from build123d import *

# Parameters (mm, degrees)
SKETCH_1_W          = 130
SKETCH_1_H          = 130
EXTRUDE_1_DEPTH     = 8
SKETCH_2_W          = 116
SKETCH_2_H          = 116
EXTRUDE_2_DEPTH     = 54
SKETCH_3_W          = 114.015684478
SKETCH_3_H          = 114.394474128
CUT_EXTRUDE_1_DEPTH = 2


with BuildPart() as part:
    # 草图1 → 凸台-拉伸1 (new body)
    with BuildSketch(Plane(origin=(0, 0, 0), x_dir=(0, 0, -1), z_dir=(1, 0, 0))):
        Rectangle(SKETCH_1_W, SKETCH_1_H)
    extrude(amount=EXTRUDE_1_DEPTH)

    # 草图2 → 凸台-拉伸2 (add)
    with BuildSketch(Plane(origin=(8, 0, 0), x_dir=(0, 0, -1), z_dir=(1, 0, 0))):
        Rectangle(SKETCH_2_W, SKETCH_2_H)
    extrude(amount=EXTRUDE_2_DEPTH)

    # 草图3 → 切除-拉伸1 (cut)
    with BuildSketch(Plane.ZY):
        Rectangle(SKETCH_3_W, SKETCH_3_H)
    extrude(amount=-CUT_EXTRUDE_1_DEPTH, mode=Mode.SUBTRACT)


solid = part.part
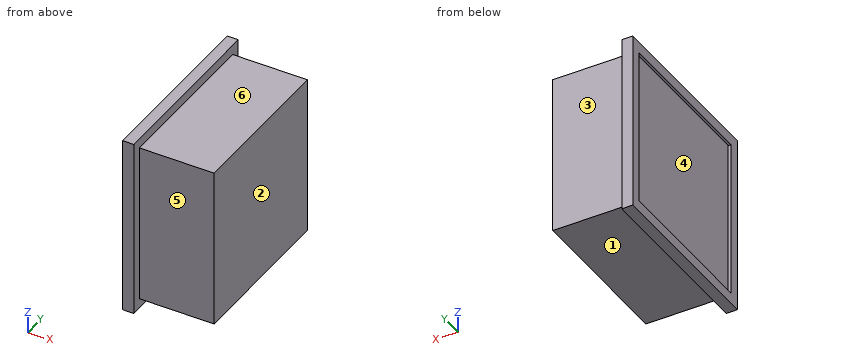
Here's how the part is built. I have some questions about the finished solid (model axes, mm). Face numbers are marked on the shaded views. A direction names the side the tool comes from. Coordinates: 2 decimals unless noted, no trailing zeros. Order: outer loops, then holes, each group sorted by start corner. A loop starts at its lowest first (then second) coordinate and runs counter-clockwise, first axis right, second up. Notation, with made-up numbers: M 83,59.5 L 131,59.5 A22 ccw 131,83.5 Z; hole C 30.5,71.25 d6. An arc over 180 degrees is marked long. Answer as CSV lines item,"result".
Item 1: If I drill on line 1 (Y direction, x = 32, z = -12.5); line 2 (X direction, y = 42, z = 32.5), over which ranges is the centre line in solid material (lowest first)?
Results found:
line 1,"-58 to 58"
line 2,"2 to 62"
Item 2: Imagine slicing it at C-C on x = 31. Write out the boundary of the cut face in (y, z), plus the area to 3 significant figures.
Results found:
outline,"M -58,-58 L 58,-58 L 58,58 L -58,58 Z"
area,"13,500 mm2"
Item 3: Imagine slicing it at B-B on y = 23.5. Write out the boundary of the cut face in (x, z), plus the area to 3 significant figures.
Results found:
outline,"M 0,-65 L 8,-65 L 8,-58 L 62,-58 L 62,58 L 8,58 L 8,65 L 0,65 L 0,57.01 L 2,57.01 L 2,-57.01 L 0,-57.01 Z"
area,"7,080 mm2"
Item 4: Imagine slicing it at A-A on z = 7. Write out the boundary of the cut face in (x, y).
Results found:
outline,"M 0,-65 L 8,-65 L 8,-58 L 62,-58 L 62,58 L 8,58 L 8,65 L 0,65 L 0,57.2 L 2,57.2 L 2,-57.2 L 0,-57.2 Z"
Item 5: We'd pull the mould along Z, two halves only. Please class the marked faces 4, 5 and 6: +Z half, -Z half, draft (parallel to the pull), parting line (faces both ways), or undercut.
Results found:
face 4,"undercut"
face 5,"draft"
face 6,"+Z half"
Item 6: For pin 1 (10 mm diameter, centred on x = 21, z = -11, fed in from +Y); pin 2 (3 mm diameter, centred on x = 55, y = -10, fed in from +Z); pin 3 (2 mm diameter, centred on y = -5.5, z = -5.5, fed in from -X), each with a flat end and sliding along its axis, tell me the tip position at first contact or that it passes through.
Results found:
pin 1,"y = 58"
pin 2,"z = 58"
pin 3,"x = 2"
Item 7: On a 3-axis mill with a long thin cutter (end or side, diameter ignored), from which of +Z, -Z, +X, -X, +Y, -Y can I reach the whole of each face in a straight line? I mean the marked faces 1, 2 and 3. Say none if no direction works.
Results found:
face 1,"-Z, +X, +Y, -Y"
face 2,"+Z, -Z, +X, +Y, -Y"
face 3,"+Z, -Z, +X, +Y"
